from build123d import *

# Parameters (mm, degrees)
SKETCH1_W           = 270
SKETCH1_H           = 270
SKETCH1_W_2         = 250
SKETCH1_H_2         = 250
EXTRUDE_THIN1_DEPTH = 800


with BuildPart() as part:
    # Sketch1 → Extrude-Thin1 (new body)
    with BuildSketch(Plane.XY):
        Rectangle(SKETCH1_W, SKETCH1_H)
        Rectangle(SKETCH1_W_2, SKETCH1_H_2, mode=Mode.SUBTRACT)
    extrude(amount=EXTRUDE_THIN1_DEPTH)


solid = part.part
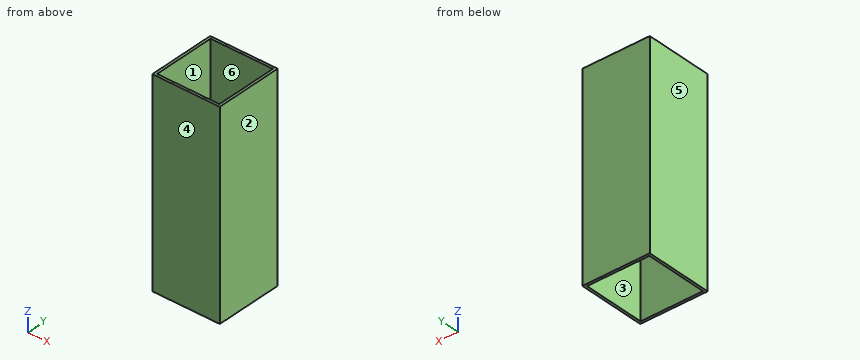
Geometry check sheet. Reference: the model listing, model coordinates, mm. Face numbers are marked on the shaded views. A direction names the side the tool comes from. Give positions to 0.01 mm unless a question says otherwise; leave off trailing zeros. Loops run counter-clockwise (first coordinate to the right, second up) from the corner with the lowest first, then second, coordinate; pieces in that order, holes last. Notation, with made-up numbers: M -16.75,-7 L -1.75,-7 A15 cw -1.75,-1 Z; hole C 70.25,1.5 d6. An arc over 180 degrees is marked long. Answer as a JSON object with one key per item and string values. Group by question number.
Item 1: Access from +Z, -Z, +X, -X, +Y, -Y to the whole of each face (thin tool, end or side, straight path). Record for the marked faces 5 and 6.
Item 2: Sectioned sample at A-A on x = 2. Record the boundary of the cut face in (y, z).
Item 3: Material ranges on L1, parallel to Y at x = -19, z = 77, recorded low to high.
Item 4: Mould release check, pull along Y, two halves, no side actions. Record for the marked faces 1, 2, 3 and 4: pulls with the +Y half, pulls with the -Y half, needs draft (parallel to the pull), parting line crosses it, or undercut.
Item 5: Sectioned sample at C-C on z = 346. Record the boundary of the cut face in (x, y), plus the area to 3 significant figures.
Findings below:
{
 "1": {"face 5": "+Z, -Z, -X, +Y, -Y", "face 6": "+Z, -Z"},
 "2": {"outline": "M -135,0 L -125,0 L -125,800 L -135,800 Z; M 125,0 L 135,0 L 135,800 L 125,800 Z"},
 "3": {"L1": "-135 to -125, 125 to 135"},
 "4": {"face 1": "undercut", "face 2": "needs draft", "face 3": "undercut", "face 4": "pulls with the -Y half"},
 "5": {"outline": "M -135,-135 L 135,-135 L 135,135 L -135,135 Z; hole M -125,-125 L 125,-125 L 125,125 L -125,125 Z", "area": "10,400 mm2"}
}
